Work out the finished part from the listing and answer in its coordinate system (mm). Coordinates: 2 decimals unless noted, no trailing zeros. Loops run counter-clockwise (first coordinate to the right, second up) from the corner with the lowest first, then second, coordinate; pieces in that order, holes last. Notation, with made-up numbers: (17.5, -38.5) -> (31.5, -38.5) arc R20 ccw to (31.5, -8.5) -> close; hole circle Ø7 at (37.25, 50). An arc over 180 degrees is marked (long way). One line per question, with ' | ' between items.
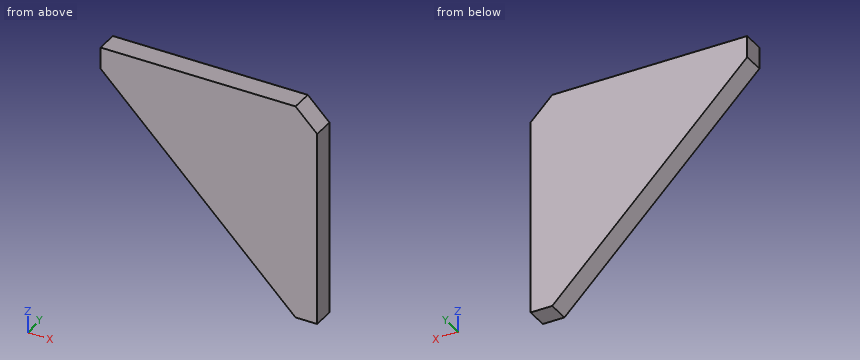
```python
from build123d import *

# Parameters (mm, degrees)
EXTRUDE_1_DEPTH = 20


with BuildPart() as part:
    # 草图1 → 凸台-拉伸1 (new body)
    with BuildSketch(Plane(origin=(0, 0, 0), x_dir=(1, 0, 0), z_dir=(0, 1, 0))):
        Polygon((0, 0), (0, -180), (-20, -200), (-200, -200), (-200, -180), (-20, 0), align=None)
    extrude(amount=EXTRUDE_1_DEPTH)


solid = part.part
```
1) Find section A-A (y = 13.5). Write down the section's boundary in (x, z), plus the area to 3 significant figures.
Check values:
outline: (-200, 180) -> (-20, 0) -> (0, 0) -> (0, 180) -> (-20, 200) -> (-200, 200) -> close | area: 23,600 mm^2
2) Find section C-C (x = -122). Write down the section's boundary in (y, z), plus the area to 3 significant figures.
Check values:
outline: (0, 102) -> (20, 102) -> (20, 200) -> (0, 200) -> close | area: 1,960 mm^2
3) Find the intervals of material crossed by line 1 along X through (y, z) = (16.5, 146); line 2 along Z through (x, y) = (-69, 7); line 3 along X through (y, z) = (9.5, 181.5), in increasing order.
Check values:
line 1: x = -166 to 0 | line 2: z = 49 to 200 | line 3: x = -200 to -1.5
4) Flat-ended cylindrical pins translate along their axes: pin 1 (6 mm diameter, centred on y = 4.5, z = 163.5, fed in from -X); pin 2 (10 mm diameter, centred on y = 18, z = 86, fed in from -X); pin 3 (5 mm diameter, centred on y = 15, z = 106.5, fed in from -X). Find the tip coordinate at first contact, or state that the pin passes through.
Check values:
pin 1: stops at x = -186.5 | pin 2: stops at x = -111 | pin 3: stops at x = -129
5) Find section B-B (z = 134.5). Write down the section's boundary in (x, y), plus the area to 3 significant figures.
Check values:
outline: (-154.5, 0) -> (0, 0) -> (0, 20) -> (-154.5, 20) -> close | area: 3,090 mm^2
